from build123d import *

# Parameters (mm, degrees)
SKETCH1_R           = 10
BOSS_EXTRUDE1_DEPTH = 20
SKETCH2_R           = 8.5
BOSS_EXTRUDE2_DEPTH = 12.8
SKETCH3_R           = 4
BOSS_EXTRUDE3_DEPTH = 30
CUT_EXTRUDE1_DEPTH  = 1.2


with BuildPart() as part:
    # Sketch1 → Boss-Extrude1 (new body)
    with BuildSketch(Plane(origin=(0, 0, 0), x_dir=(1, 0, 0), z_dir=(0, 1, 0))):
        with Locations(Location((0, 0, 0), (0, 0, 270))):
            Circle(SKETCH1_R)
    extrude(amount=BOSS_EXTRUDE1_DEPTH)

    # Sketch2 → Boss-Extrude2 (add)
    with BuildSketch(Plane(origin=(0, 20, 0), x_dir=(1, 0, 0), z_dir=(0, 1, 0))):
        with Locations(Location((0, 0, 0), (0, 0, 270))):
            Circle(SKETCH2_R)
    extrude(amount=BOSS_EXTRUDE2_DEPTH)

    # Sketch3 → Boss-Extrude3 (add)
    with BuildSketch(Plane(origin=(0, 32.8, 0), x_dir=(1, 0, 0), z_dir=(0, 1, 0))):
        with Locations(Location((0, 0, 0), (0, 0, 270))):
            Circle(SKETCH3_R)
    extrude(amount=BOSS_EXTRUDE3_DEPTH)

    # Sketch4 → Cut-Extrude1 (cut)
    with BuildSketch(Plane(origin=(0, 0, -4), x_dir=(-1, 0, 0), z_dir=(0, 0, -1))):
        with BuildLine():
            Line((1, 49.8), (1, 35.8))
            ThreePointArc((1, 35.8), (0, 34.8), (-1, 35.8))
            Line((-1, 35.8), (-1, 49.8))
            ThreePointArc((-1, 49.8), (0, 50.8), (1, 49.8))
        make_face()
    extrude(amount=-CUT_EXTRUDE1_DEPTH, mode=Mode.SUBTRACT)


solid = part.part
The model under review builds one solid part; all positions refer to its coordinate system, in mm. A direction names the side the tool comes from. Round coordinates to 2 decimals unless told otherwise and drop trailing zeros. Loops run counter-clockwise (first coordinate to the right, second up) from the corner with the lowest first, then second, coordinate; pieces in that order, holes last. Notation, with made-up numbers: (72.25, 64) -> (103.25, 64) arc R14 cw to (103.25, 68) -> close; hole circle Ø4 at (3.25, 55). An arc over 180 degrees is marked (long way). Write item = value, one per line. Start each with the question number.
Item 1: Take a section at A-A on z = 0. Give the boundary of the cut face in (x, y).
Item 2: For faces 1 (the flat face through (1, 43, -3)), 2 (the flat face through (-2, 32.8, 4)), 3 (the cylindrical face through (-9.76, 9.86, -2.17)), list the 3-axis set-ups (+Z, -Z, +X, -X, +Y, -Y) from which the entire face can be reached by the end or side of a thin tool; tool diameter is ignored.
Item 3: Insertion check: pin 1 (6 mm diameter, centred on x = 4.5, z = 1, fed in from +Y); pin 2 (4 mm diameter, centred on y = 39, z = 0.5, fed in from -X); pin 3 (0.9 mm diameter, centred on y = 43.5, z = -3, fed in from +X); pin 4 (5 mm diameter, centred on x = 2.5, y = 28.5, fed in from -Z). Each pin has a flat end and moves straight along its axis. Give the tip position at first contact, or say it passes through.
Item 4: Mouldability with a two-part tool opening along X and no side actions: class faces 4 (the cylindrical face through (-1.532, 47.59, 3.695)), 5 (the flat face through (-1, 43, -3)), 6 (the flat face through (0, 43, -2.8)), 7 (the flat face through (0, 62.8, 0)) as released by +X, released by -X, zero draft, split by the parting line, or undercut.
Item 5: Take a section at D-D on y = 7.5. Give the boundary of the cut face in (x, z).
Item 6: Take a section at C-C on x = 6.5. Give the boundary of the cut face in (y, z), plus the area to 3 significant figures.
Item 7: To check wall thickness, follow L1, parallel to Y at x = -5.75, z = 4.25; L2, parallel to Y at x = -8.5, z = -2.75; L3, parallel to X at y = 30, z = -7. State the ranges of each line that lie inside material, in increasing order.
Item 8: Take a section at B-B on y = 57. Give the boundary of the cut face in (x, z).
Result:
q1.outline = (-10, 0) -> (10, 0) -> (10, 20) -> (8.5, 20) -> (8.5, 32.8) -> (4, 32.8) -> (4, 62.8) -> (-4, 62.8) -> (-4, 32.8) -> (-8.5, 32.8) -> (-8.5, 20) -> (-10, 20) -> close
q2.face_1 = -Z
q2.face_2 = +Y
q2.face_3 = +Y, -Y
q3.pin_1 = 62.8
q3.pin_2 = -4
q3.pin_3 = 3.08
q3.pin_4 = -8.5
q4.face_4 = split by the parting line
q4.face_5 = undercut
q4.face_6 = undercut
q4.face_7 = zero draft
q5.outline = circle Ø20 at (0, 0)
q6.outline = (0, -7.6) -> (20, -7.6) -> (20, -5.48) -> (32.8, -5.48) -> (32.8, 5.48) -> (20, 5.48) -> (20, 7.6) -> (0, 7.6) -> close
q6.area = 444 mm²
q7.L1 = 0 to 32.8
q7.L2 = 0 to 20
q7.L3 = -4.82 to 4.82
q8.outline = circle Ø8 at (0, 0)
